Could you check a few things on this model? Use its own coordinates, in mm. A direction names the side the tool comes from. Round coordinates to 2 decimals unless told otherwise and drop trailing zeros. Loops run counter-clockwise (first coordinate to the right, second up) from the corner with the lowest first, then second, coordinate; pieces in that order, holes last. Notation, with made-up numbers: (-37.75, 10.5) -> (-16.75, 10.5) arc R36 cw to (-16.75, 44.5) -> close; hole circle Ø6 at (86, 31). An arc over 180 degrees is marked (long way). Write each question's results on one line, items separated by ' | '. Start each with the question number.
1) Which directions (+Z, -Z, +X, -X, +Y, -Y) give clear straight access to the entire face, cutting with the end or side of a thin tool? Please do faces 1 (the flat face through (-13, -6, 17)), 2 (the cylindrical face through (-19.5, 0.07, 18.48)).
2) If I drill on probe 1 along Y at (x, z) = (0, 18.1); probe 2 along Y at (x, z) = (0, -5.5); probe 3 along Z at (x, y) = (15.5, 6.5), over which ranges is the centre line in solid material (lowest first)?
3) Imagine slicing it at D-D, the plane x = -4. List the corners of the cut face in (y, z) for me.
4) Imagine slicing it at C-C, the plane z = 19. List the corners of the cut face in (x, y) for me.
5) We'd pull the mould along X, two halves only. Please class faces 3 (the flat face through (-13, -6, 20)), 4 (the cylindrical face through (12.932, -5.362, 22.535)), 5 (the cylindrical face through (11.923, 3.755, -0.35)): pulls with the +X half, pulls with the -X half, needs draft (parallel to the pull), parting line crosses it, or undercut.
6) Imagine slicing it at B-B, the plane y = 18. List the corners of the cut face in (x, z) for me, plus the area to 3 significant figures.
7) For P1, Ø5, axis at x = 18, y = 0, coming from the -Z side; P2, Ø4, axis at y = 1.5, z = -6, coming from the +X side; P3, Ø1, axis at x = 13.5, y = -9, coming from the +Z side, each with a flat end and sliding along its axis, tell me the tip position at first contact or that it passes through.
8) Imagine slicing it at A-A, the plane x = 0. List the corners of the cut face in (y, z) for me, plus the area to 3 significant figures.
from build123d import *

# Parameters (mm, degrees)
SKETCH1_R           = 14
SKETCH1_R_2         = 12.5
BOSS_EXTRUDE1_DEPTH = 25
BOSS_EXTRUDE2_START = -8
SKETCH2_R           = 20
SKETCH2_R_2         = 1.5
SKETCH2_R_3         = 12.5
BOSS_EXTRUDE2_DEPTH = 3


with BuildPart() as part:
    # Sketch1 → Boss-Extrude1 (new, symmetric)
    with BuildSketch(Plane.XY):
        Circle(SKETCH1_R)
        Circle(SKETCH1_R_2, mode=Mode.SUBTRACT)
    extrude(amount=BOSS_EXTRUDE1_DEPTH, both=True)

    # Sketch2 → Boss-Extrude2 (add)
    with BuildSketch(Plane.XY.offset(25).offset(BOSS_EXTRUDE2_START)):
        Circle(SKETCH2_R)
        with Locations((0, 18)):
            Circle(SKETCH2_R_2, mode=Mode.SUBTRACT)
        with Locations((18, 0)):
            Circle(SKETCH2_R_2, mode=Mode.SUBTRACT)
        with Locations((0, -18)):
            Circle(SKETCH2_R_2, mode=Mode.SUBTRACT)
        with Locations((-18, 0)):
            Circle(SKETCH2_R_2, mode=Mode.SUBTRACT)
        Circle(SKETCH2_R_3, mode=Mode.SUBTRACT)
    extrude(amount=BOSS_EXTRUDE2_DEPTH)


solid = part.part
Checked values:
1) face 1: -Z | face 2: +Z, -Z
2) probe 1: -20 to -19.5, -16.5 to -12.5, 12.5 to 16.5, 19.5 to 20 | probe 2: -14 to -12.5, 12.5 to 14 | probe 3: 17 to 20
3) outline: (-19.6, 17) -> (-13.42, 17) -> (-13.42, -25) -> (-11.84, -25) -> (-11.84, 25) -> (-13.42, 25) -> (-13.42, 20) -> (-19.6, 20) -> close; (11.84, -25) -> (13.42, -25) -> (13.42, 17) -> (19.6, 17) -> (19.6, 20) -> (13.42, 20) -> (13.42, 25) -> (11.84, 25) -> close
4) outline: circle Ø40 at (0, 0); hole circle Ø3 at (-18, 0); hole circle Ø25 at (0, 0); hole circle Ø3 at (0, -18); hole circle Ø3 at (0, 18); hole circle Ø3 at (18, 0)
5) face 3: needs draft | face 4: parting line crosses it | face 5: undercut
6) outline: (-8.72, 17) -> (-1.5, 17) -> (-1.5, 20) -> (-8.72, 20) -> close; (1.5, 17) -> (8.72, 17) -> (8.72, 20) -> (1.5, 20) -> close | area: 43.3 mm^2
7) P1: z = 17 | P2: x = 14 | P3: z = 20
8) outline: (-20, 17) -> (-19.5, 17) -> (-19.5, 20) -> (-20, 20) -> close; (-16.5, 17) -> (-14, 17) -> (-14, -25) -> (-12.5, -25) -> (-12.5, 25) -> (-14, 25) -> (-14, 20) -> (-16.5, 20) -> close; (12.5, -25) -> (14, -25) -> (14, 17) -> (16.5, 17) -> (16.5, 20) -> (14, 20) -> (14, 25) -> (12.5, 25) -> close; (19.5, 17) -> (20, 17) -> (20, 20) -> (19.5, 20) -> close | area: 168 mm^2
